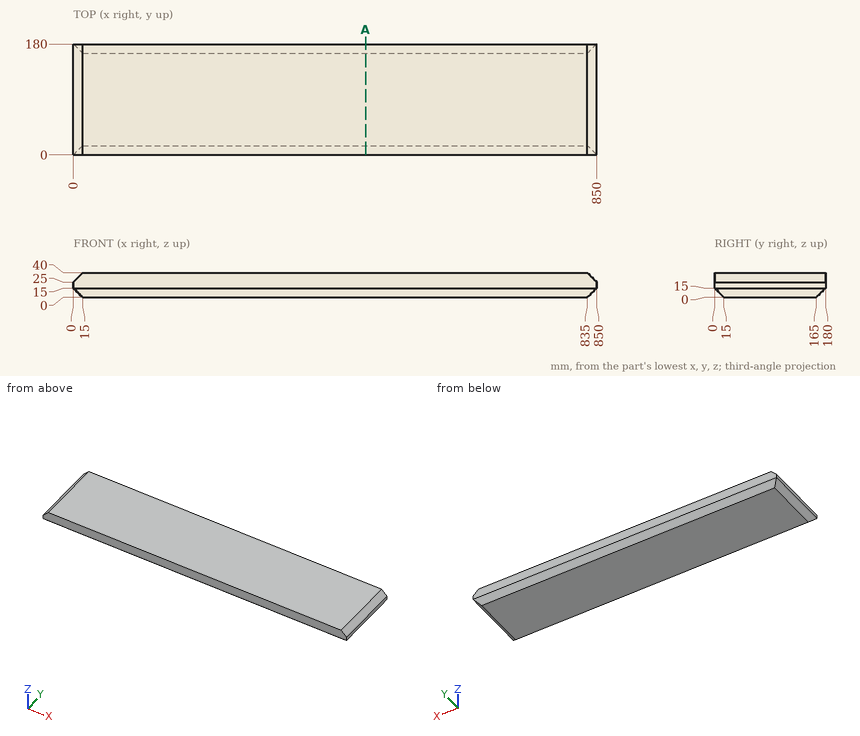
The drawing under review shows one solid part. Ordinate dimensions are in mm from its lowest x, y, z. Round coordinates to 2 decimals unless told otherwise and drop trailing zeros. Write each loop counter-clockwise with the first axis right and the second up, starting at its lowest first coordinate (ties: lowest second). Pieces come first, ordered by that corner, then holes. Notation, with made-up numbers: (-12, -9.5) - (-7, -9.5) arc R24 ccw to (-7, 23.5) - close; hole circle Ø3 at (4.25, -9). An arc over 180 degrees is marked (long way). Put each result on its own line as item: value.
Q1. Insertion check: pin 1 Ø10 at (x, z) = (566.5, 8) entering from +Y; pin 2 Ø3 at (y, z) = (87.5, 31) entering from -X; pin 3 Ø1 at (y, z) = (25, 31) entering from +X. Each pin has a flat end and moves straight along its axis. Give the tip position at first contact, or say it passes through.
Solved:
pin 1: stops at y = 178
pin 2: stops at x = 4.5
pin 3: stops at x = 844.5
Q2. Wall thickness on probe 1 along X at (y, z) = (141.5, 8.5); probe 2 along Y at (x, z) = (379, 14); probe 3 along Y at (x, z) = (702.5, 6): over which ranges is each line inside the solid? List them lowest first.
Solved:
probe 1: x = 6.5 to 843.5
probe 2: y = 1 to 179
probe 3: y = 9 to 171
Q3. We need section A-A (x = 474.5). Give the boundary of the cut face in (y, z).
Solved:
outline: (0, 15) - (15, 0) - (165, 0) - (180, 15) - (180, 40) - (0, 40) - close
